Input: part model. Units: mm. Frame: model coordinates. A direction names the side the tool comes from. Coordinates: 2 decimals unless noted, no trailing zeros. Loops run counter-clockwise (first coordinate to the right, second up) from the corner with the lowest first, then second, coordinate; pieces in that order, holes last. Notation, with made-up numbers: (67.25, 21) - (77.25, 21) arc R10 cw to (77.25, 30) - close; hole circle Ø7 at (72, 62). An arc over 180 degrees is marked (long way). Use a Markdown table: item, result. Add a question column.
1. Access query for faces 4 (the face through (-138.395, -9.348, 80.892)), 5 (the face through (-127, -25, 0)), 6 (the face through (-135.93, 7.65, 61.8)). Directions: +Z, -Z, +X, -X, +Y, -Y. A direction counts if a zero-diameter tool reaches every point of the face in a straight line with its end or side. Return the directions, or none.
2. Ray query, L1, parallel to Y at x = -143, z = 12; L2, parallel to Y at x = -131, z = 65.5; L3, parallel to Z at x = -122.5, y = -8. Return the intervals inside material, ascending. Write a range as [from, to].
3. Section query D-D on y = -33. Return the cut outline in (x, z), then the cut area to 3 significant figures.
4. Contact query for flat-ended pins moving along their axis: P1, Ø2, axis at x = -151, y = -36.5, coming from the +Z side; P2, Ø1, axis at x = -133, y = 8.5, coming from the -Z side; P3, Ø2, axis at x = -129.5, z = 44.5, coming from the -Y side. Output: stop coordinate, or through.
5. Draft query along X for faces 1 (the face through (-163.045, -6.9, 80.1)), 2 (the face through (-137, 0, 84)), 3 (the face through (-143.46, -38.26, 19.09)). Return one class per face: released by +X, released by -X, zero draft, split by the parting line, or undercut.
6. Section query A-A on y = -22. Return the cut outline in (x, z).
7. Section query C-C on z = 71. Return the cut outline in (x, y).
8. Section query B-B on x = -118. Return the cut outline in (y, z).
```python
from build123d import *

# Parameters (mm, degrees)
SKETCH1_R           = 25
BOSS_EXTRUDE1_DEPTH = 50
SKETCH3_R           = 29.577748383
BOSS_EXTRUDE2_DEPTH = 25
SKETCH4_R           = 15
BOSS_EXTRUDE3_DEPTH = 5
CUT_EXTRUDE1_REACH  = 118.762
SKETCH5_R           = 15
SKETCH6_R           = 1.5
CUT_EXTRUDE2_DEPTH  = 20


with BuildPart() as part:
    # Sketch1 → Boss-Extrude1 (new body)
    with BuildSketch(Plane.XY):
        with Locations((-138.044677266, -13.853162466)):
            Circle(SKETCH1_R)
    extrude(amount=BOSS_EXTRUDE1_DEPTH)

    # Sketch3 → Boss-Extrude2 (add, symmetric)
    with BuildSketch(Plane(origin=(-138.044677266, 0, 0), x_dir=(0, 0, -1), z_dir=(1, 0, 0))):
        with Locations((-66.584372838, -13.853162466)):
            Circle(SKETCH3_R)
    extrude(amount=BOSS_EXTRUDE2_DEPTH, both=True)

    # Sketch4 → Boss-Extrude3 (add, symmetric)
    with BuildSketch(Plane(origin=(0, 0, 0), x_dir=(-1, 0, 0), z_dir=(0, 0, -1))):
        with Locations(Location((138.044677266, -13.853162466, 0), (0, 0, 180))):
            Circle(SKETCH4_R)
    extrude(amount=BOSS_EXTRUDE3_DEPTH, both=True)

    # Sketch5 → Cut-Extrude1 (cut, up to next)
    with BuildSketch(Plane.ZY.offset(163.044677266), mode=Mode.PRIVATE) as cut_extrude1_sk1:
        with Locations((66.584372838, -13.853162466)):
            Circle(SKETCH5_R)
    cut_extrude1_tool1 = extrude(cut_extrude1_sk1.sketch, amount=-CUT_EXTRUDE1_REACH, mode=Mode.PRIVATE) & part.part
    add(cut_extrude1_tool1.solids().sort_by_distance((-163.044677, -13.853162, 66.584373))[0], mode=Mode.SUBTRACT)

    # Sketch6 → Cut-Extrude2 (cut)
    with BuildSketch(Plane(origin=(0, 0, 0), x_dir=(1, 0, 0), z_dir=(0, 1, 0))):
        with Locations(Location((-137.396937397, -61.478842375, 0), (0, 0, 90))):
            Circle(SKETCH6_R)
        with Locations(Location((-137.396937397, -83.561946624, 0), (0, 0, 90))):
            Circle(SKETCH6_R)
    extrude(amount=CUT_EXTRUDE2_DEPTH, mode=Mode.SUBTRACT)


solid = part.part
```
Resolved:
| question | item | result |
|---|---|---|
| 1 | face 4 | +X, -X |
| 1 | face 5 | -Z |
| 1 | face 6 | +Y |
| 2 | L1 | [-38.36, 10.65] |
| 2 | L2 | [-43.41, -28.81], [1.11, 15.7] |
| 2 | L3 | [0, 52.77], [80.4, 95.58] |
| 3 | outline | (-163.04, 44.04) - (-154.12, 44.04) - (-154.12, 0) - (-121.97, 0) - (-121.97, 44.04) - (-113.04, 44.04) - (-113.04, 89.13) - (-163.04, 89.13) - close |
| 3 | area | 3,670 mm² |
| 4 | P1 | z = 86.74 |
| 4 | P2 | z = 0 |
| 4 | P3 | y = -37.69 |
| 5 | face 1 | released by -X |
| 5 | face 2 | undercut |
| 5 | face 3 | split by the parting line |
| 6 | outline | (-163.04, 38.15) - (-161.68, 38.15) - (-161.68, 0) - (-150.64, 0) - (-150.64, -5) - (-125.45, -5) - (-125.45, 0) - (-114.41, 0) - (-114.41, 38.15) - (-113.04, 38.15) - (-113.04, 53.99) - (-163.04, 53.99) - close; (-163.04, 79.18) - (-113.04, 79.18) - (-113.04, 95.02) - (-163.04, 95.02) - close |
| 7 | outline | (-163.04, -43.1) - (-113.04, -43.1) - (-113.04, -28.19) - (-163.04, -28.19) - close; (-163.04, 0.48) - (-113.04, 0.48) - (-113.04, 15.39) - (-163.04, 15.39) - close |
| 8 | outline | (-28.79, 0) - (1.09, 0) - (1.09, 41.06) arc R29.58 ccw (long way) to (-28.79, 41.06) - close; hole circle Ø30 at (-13.85, 66.58) |
